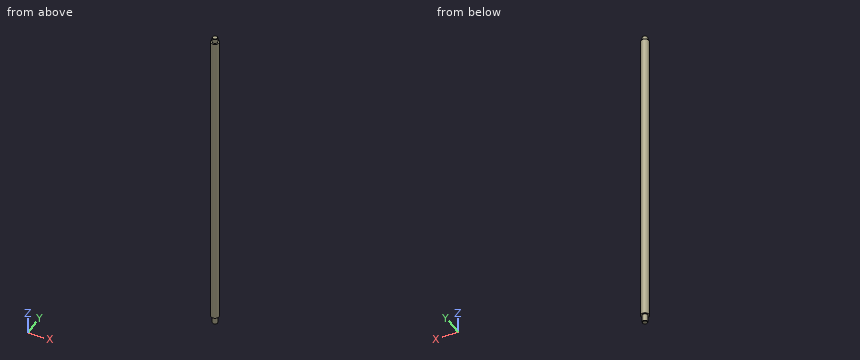
from build123d import *

# Parameters (mm, degrees)
SKETCH_1_R        = 12.5
EXTRUDE_210_DEPTH = 990
SKETCH_2_R        = 8
EXTRUDE_1_DEPTH   = 15
EXTRUDE_START     = 25
SKETCH_3_R        = 8
EXTRUDE_2_DEPTH   = 25
CHAMFER_1_SIZE    = 1


with BuildPart() as part:
    # 草图1 → Extrude 210 (new body)
    with BuildSketch(Plane.XY):
        Circle(SKETCH_1_R)
    extrude(amount=EXTRUDE_210_DEPTH)

    # 草图2 → 凸台-拉伸1 (add)
    with BuildSketch(Plane.XY.offset(990)):
        Circle(SKETCH_2_R)
    extrude(amount=EXTRUDE_1_DEPTH)

    # 草图3 → 凸台-拉伸2 (add)
    with BuildSketch(Plane(origin=(0, 0, 0), x_dir=(-1, 0, 0), z_dir=(0, 0, -1)).offset(EXTRUDE_START)):
        with Locations(Location((0, 0, 0), (0, 0, 180))):
            Circle(SKETCH_3_R)
    extrude(amount=-EXTRUDE_2_DEPTH)

    # 倒角1
    chamfer_1_edges = [part.edges().sort_by_distance(p)[0] for p in [
        (-8, 0, 1005),
        (-8, 0, -25),
    ]]
    chamfer(chamfer_1_edges, length=CHAMFER_1_SIZE)


solid = part.part
The listing builds one solid part. Answer for the finished solid, in the listing's coordinates (mm). Coordinates: 2 decimals unless noted, no trailing zeros. Write each loop counter-clockwise with the first axis right and the second up, starting at its lowest first coordinate (ties: lowest second). Pieces come first, ordered by that corner, then holes. Notation, with made-up numbers: (38, 20) - (87, 20) arc R20 ccw to (87, 56) - close; hole circle Ø3 at (-33, 41.5). An arc over 180 degrees is marked (long way). Return JSON: item names as keys, results as strings.
1. Consider line 1 along Z through (x, y) = (-3, 8.5); line 2 along X through (y, z) = (-10.25, 582.5); line 3 along Y through (x, z) = (1, 450). Determine where each line is inside the solid, lowest interval first.
Final values:
{"line 1": "0 to 990", "line 2": "-7.15 to 7.15", "line 3": "-12.46 to 12.46"}
2. Each of these flat-tipped pins is pushed along its axis until it touches: pin 1 Ø8 at (x, z) = (6.5, 489) entering from +Y; pin 2 Ø1 at (y, z) = (5, 216.5) entering from +X; pin 3 Ø1 at (y, z) = (9.5, 323.5) entering from +X; pin 4 Ø1 at (x, z) = (0.5, 200) entering from +Y. Where does it stop, or does it pass through?
Final values:
{"pin 1": "y = 12.25", "pin 2": "x = 11.66", "pin 3": "x = 8.67", "pin 4": "y = 12.5"}
3. The part is cut by section A-A on z = 224. Determine the outline of the cut face in (x, y).
Final values:
{"outline": "circle Ø25 at (0, 0)"}
